The listing builds one solid part. Answer for the finished solid, in the listing's coordinates (mm). Face numbers are marked on the shaded views. A direction names the side the tool comes from. Give positions to 0.01 mm unless a question says otherwise; leave off trailing zeros. Order: outer loops, then holes, each group sorted by start corner. A loop starts at its lowest first (then second) coordinate and runs counter-clockwise, first axis right, second up. Notation, with made-up numbers: (8, 9.25) - (30, 9.25) arc R7 cw to (30, 20.25) - close; hole circle Ø6 at (70, 82). An arc over 180 degrees is marked (long way). Use a Markdown table: item, result. Add a question column.
1) For the marked faces 4, 5 and 6, determine the directions among +Z, -Z, +X, -X, +Y, -Y from which every point of the face is accessible in a straight line to the end or side of a thin tool.
2) Flat-ended cylindrical pins translate along their axes: pin 1 (3 mm diameter, centred on x = 79, z = -17, fed in from +Y); pin 2 (12 mm diameter, centred on x = 6.5, y = 21.5, fed in from -Z); pin 3 (9 mm diameter, centred on x = 80, z = -13, fed in from -Y); pin 4 (11 mm diameter, centred on x = 8.5, y = 6, fed in from -Z). Find the tip coordinate at first contact, or state that the pin passes through.
3) Find section B-B, the plane x = 61.5. Determine the outline of the cut face in (y, z).
4) Find section A-A, the plane y = 32. Determine the outline of the cut face in (x, z).
5) Straight lines are drawn through the part: line 1 (X direction, y = 2, z = -13); line 2 (Y direction, x = 18.5, z = -25); line 3 (X direction, y = 7, z = -21). For each, find the intervals that lie inside material, in ascending order.
6) The mould has two halves that part along X. Classify the marked faces 1, 2 and 3: released by +X, released by -X, zero draft, split by the parting line, or undercut.
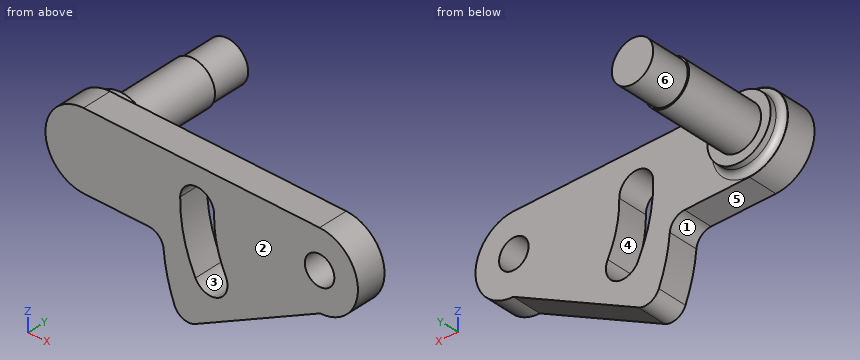
from build123d import *

# Parameters (mm, degrees)
SKETCH_1_R      = 5
EXTRUDE_1_DEPTH = 10
FILLET_2_R      = 5
SKETCH_2_R      = 10.75
EXTRUDE_2_DEPTH = 4
FILLET_3_R      = 2
SKETCH_3_R      = 7.5
EXTRUDE_3_DEPTH = 27
SKETCH_5_R      = 7
EXTRUDE_4_DEPTH = 13


with BuildPart() as part:
    # 草图1 → 凸台-拉伸1 (new body)
    with BuildSketch(Plane(origin=(0, 0, 0), x_dir=(1, 0, 0), z_dir=(0, 1, 0))):
        with BuildLine():
            Line((0, 0), (80, 0))
            ThreePointArc((80, 0), (92.999656788, 12.905536238), (80.188922536, 25.998627169))
            Line((80.188922536, 25.998627169), (33.171963216, 50.997987887))
            ThreePointArc((33.171963216, 50.997987887), (28.520841175, 38.881634135), (26.938922553, 26))
            Line((26.938922553, 26), (0.188922547, 26))
            ThreePointArc((0.188922547, 26), (-12.905538726, 13.094461274), (0, 0))
        make_face()
        with Locations(Location((80, 13, 0), (0, 0, 270))):
            Circle(SKETCH_1_R, mode=Mode.SUBTRACT)
        with BuildLine():
            ThreePointArc((48.162206807, 29.260917091), (45.167661271, 21.048023276), (44.255838588, 12.353915663))
            ThreePointArc((44.255838588, 12.353915663), (38.610693325, 6.500939074), (32.757716736, 12.146084337))
            ThreePointArc((32.757716736, 12.146084337), (33.962853008, 23.636897896), (37.920678927, 34.491701609))
            ThreePointArc((37.920678927, 34.491701609), (45.656835127, 36.99707329), (48.162206807, 29.260917091))
        make_face(mode=Mode.SUBTRACT)
    extrude(amount=EXTRUDE_1_DEPTH)

    # 圆角2
    fillet_2_edges = [part.edges().sort_by_distance(p)[0] for p in [
        (26.938922553, 5, -26),
        (33.171963216, 5, -50.997987887),
    ]]
    fillet(fillet_2_edges, radius=FILLET_2_R)

    # 草图2 → 凸台-拉伸2 (add)
    with BuildSketch(Plane(origin=(0, 10, 0), x_dir=(1, 0, 0), z_dir=(0, 1, 0))):
        with Locations(Location((0.094461274, 13, 0), (0, 0, 270))):
            Circle(SKETCH_2_R)
    extrude(amount=EXTRUDE_2_DEPTH)

    # 圆角3
    fillet_3_edges = [part.edges().sort_by_distance(p)[0] for p in [
        (0.094461274, 10, -23.75),
    ]]
    fillet(fillet_3_edges, radius=FILLET_3_R)

    # 草图3 → 凸台-拉伸3 (add)
    with BuildSketch(Plane(origin=(0, 14, 0), x_dir=(1, 0, 0), z_dir=(0, 1, 0))):
        with Locations(Location((0.094461274, 13, 0), (0, 0, 270))):
            Circle(SKETCH_3_R)
    extrude(amount=EXTRUDE_3_DEPTH)

    # 草图5 → 凸台-拉伸4 (add)
    with BuildSketch(Plane(origin=(0, 41, 0), x_dir=(1, 0, 0), z_dir=(0, 1, 0))):
        with Locations(Location((0.094461274, 13, 0), (0, 0, 90))):
            Circle(SKETCH_5_R)
    extrude(amount=EXTRUDE_4_DEPTH)


solid = part.part
The answers:
| question | item | result |
|---|---|---|
| 1 | face 4 | +Y, -Y |
| 1 | face 5 | -Z, -X, +Y, -Y |
| 1 | face 6 | +Y |
| 2 | pin 1 | y = 10 |
| 2 | pin 2 | z = -20.49 |
| 2 | pin 3 | through |
| 2 | pin 4 | z = -26 |
| 3 | outline | (0, -35.94) - (10, -35.94) - (10, 0) - (0, 0) - close |
| 4 | outline | circle Ø15 at (0.09, -13) |
| 5 | line 1 | -12.91 to 32.75, 44.25 to 75, 85 to 93 |
| 5 | line 2 | 0 to 10 |
| 5 | line 3 | -10.15 to 33.43, 45.16 to 90.25 |
| 6 | face 1 | released by -X |
| 6 | face 2 | zero draft |
| 6 | face 3 | undercut |
